Could you check a few things on this model? Use its own coordinates, in mm. Face numbers are marked on the shaded views. A direction names the side the tool comes from. Coordinates: 2 decimals unless noted, no trailing zeros. Order: outer loops, then holes, each group sorted by start corner. A loop starts at its lowest first (then second) coordinate and runs counter-clockwise, first axis right, second up. Notation, with made-up numbers: (44, 38.25) -> (55, 38.25) arc R17 cw to (55, 44.25) -> close; hole circle Ø1 at (40.25, -9.75). An arc over 180 degrees is marked (long way). Put each result on its own line as item: value. Start each with the question number.
Q1. Please list where these lines run through material, in increasing order: line 1 along X through (y, z) = (25, 0); line 2 along Z through (x, y) = (0, 27); line 3 along Z through (x, y) = (32.5, 40).
Q2. If we section it at A-A (x = 0): Please give me the cut outline in (y, z).
Q3. We'd pull the mould along Z, two halves only. Please class the marked faces 1, 2 and 3: +Z half, -Z half, draft (parallel to the pull), parting line (faces both ways), or undercut.
Q4. Will these pins go through, and if not, where does the flat tip stop? pin 1 (7.5 mm diameter, centred on y = 50, z = 45, fed in from -X); pin 2 (24.5 mm diameter, centred on x = -38.5, z = -24, fed in from +Y); pin 3 (7.5 mm diameter, centred on y = 51.5, z = -38, fed in from +X); pin 4 (2 mm diameter, centred on y = 25, z = -28, fed in from +X).
Q5. For the marked faces 4, 5 and 6, which set-ups out of +Z, -Z, +X, -X, +Y, -Y let a thin tool reach every point of the face, with its end or its side?
Q6. If we section it at C-C (y = 19.5): Please give me the cut outline in (x, z), and give its area (3 significant figures).
Q7. If we section it at D-D (x = 45.5): Please give me the cut outline in (y, z).
Q8. If we section it at B-B (y = 44): Count the separate pieces of the cut face and the enclosed holes in it, and give its area (3 significant figures).
from build123d import *

# Parameters (mm, degrees)
HEX_BODY_104AF_X_60_DEPTH      = 60
CROWN_CHAMFER_SKETCH_OUTSIDE_W = 276.052
CROWN_CHAMFER_SKETCH_OUTSIDE_H = 259.964
CROWN_CHAMFER_SKETCH_OUTSIDE_R = 52
CROWN_CHAMFER_45DEG_DEPTH      = 60
CROWN_CHAMFER_45DEG_DRAFT      = -45
BORE_SKETCH_50_R               = 25
BORE_50_DEPTH                  = 60
CASTLE_SLOTS_6X10_DEPTH        = 25


with BuildPart() as part:
    # Hex Profile Sketch → Hex Body 104AF x 60 (new body)
    with BuildSketch(Plane(origin=(0, 0, 0), x_dir=(1, 0, 0), z_dir=(0, 1, 0))):
        Polygon((30.022213998, -52), (60.044427996, 0), (30.022213998, 52), (-30.022213998, 52), (-60.044427996, 0), (-30.022213998, -52), align=None)
    extrude(amount=HEX_BODY_104AF_X_60_DEPTH)


with BuildPart() as crown_chamfer_45deg_tool:
    # Crown Chamfer Sketch outside → Crown Chamfer 45deg (with draft: the straight prism first)
    with BuildSketch(Plane(origin=(0, 60, 0), x_dir=(1, 0, 0), z_dir=(0, 1, 0))):
        Rectangle(CROWN_CHAMFER_SKETCH_OUTSIDE_W, CROWN_CHAMFER_SKETCH_OUTSIDE_H)
        Circle(CROWN_CHAMFER_SKETCH_OUTSIDE_R, mode=Mode.SUBTRACT)
    extrude(amount=-CROWN_CHAMFER_45DEG_DEPTH)
    # Crown Chamfer 45deg: the draft: its side faces are tilted about the plane it starts from
    crown_chamfer_45deg_sides = [crown_chamfer_45deg_tool.faces().sort_by_distance(p)[0] for p in [
        (0, 30, 129.982),
        (138.026, 30, 0),
        (0, 30, -129.982),
        (-138.026, 30, 0),
        (-52, 30, 0),
    ]]
    draft(crown_chamfer_45deg_sides, Plane(origin=(0, 60, 0), x_dir=(1, 0, 0), z_dir=(0, 1, 0)), CROWN_CHAMFER_45DEG_DRAFT)


with BuildPart() as part_1:
    add(part.part)

    # Crown Chamfer 45deg: cut by crown_chamfer_45deg_tool
    add(crown_chamfer_45deg_tool.part, mode=Mode.SUBTRACT)

    # Bore Sketch Ø50 → Bore Ø50 (cut)
    with BuildSketch(Plane(origin=(0, 60, 0), x_dir=(1, 0, 0), z_dir=(0, 1, 0))):
        with Locations(Location((0, 0, 0), (0, 0, 270))):
            Circle(BORE_SKETCH_50_R)
    extrude(amount=-BORE_50_DEPTH, mode=Mode.SUBTRACT)

    # Castle Slots Sketch → Castle Slots 6x10 (cut)
    with BuildSketch(Plane(origin=(0, 60, 0), x_dir=(1, 0, 0), z_dir=(0, 1, 0))):
        with BuildLine():
            Line((-5, -24.494897428), (-5, -52))
            Line((-5, -52), (0, -52))
            Line((0, -52), (5, -52))
            Line((5, -52), (5, -24.494897428))
            ThreePointArc((5, -24.494897428), (0, -25), (-5, -24.494897428))
        make_face()
        with BuildLine():
            Line((-23.713203436, -7.917321695), (-47.533320997, -21.669872981))
            Line((-47.533320997, -21.669872981), (-45.033320997, -26))
            Line((-45.033320997, -26), (-42.533320997, -30.330127019))
            Line((-42.533320997, -30.330127019), (-18.713203436, -16.577575733))
            ThreePointArc((-18.713203436, -16.577575733), (-21.650635095, -12.5), (-23.713203436, -7.917321695))
        make_face()
        with BuildLine():
            Line((-18.713203436, 16.577575733), (-42.533320997, 30.330127019))
            Line((-42.533320997, 30.330127019), (-45.033320997, 26))
            Line((-45.033320997, 26), (-47.533320997, 21.669872981))
            Line((-47.533320997, 21.669872981), (-23.713203436, 7.917321695))
            ThreePointArc((-23.713203436, 7.917321695), (-21.650635095, 12.5), (-18.713203436, 16.577575733))
        make_face()
        with BuildLine():
            Line((5, 24.494897428), (5, 52))
            Line((5, 52), (0, 52))
            Line((0, 52), (-5, 52))
            Line((-5, 52), (-5, 24.494897428))
            ThreePointArc((-5, 24.494897428), (0, 25), (5, 24.494897428))
        make_face()
        with BuildLine():
            Line((23.713203436, 7.917321695), (47.533320997, 21.669872981))
            Line((47.533320997, 21.669872981), (45.033320997, 26))
            Line((45.033320997, 26), (42.533320997, 30.330127019))
            Line((42.533320997, 30.330127019), (18.713203436, 16.577575733))
            ThreePointArc((18.713203436, 16.577575733), (21.650635095, 12.5), (23.713203436, 7.917321695))
        make_face()
        with BuildLine():
            Line((18.713203436, -16.577575733), (42.533320997, -30.330127019))
            Line((42.533320997, -30.330127019), (45.033320997, -26))
            Line((45.033320997, -26), (47.533320997, -21.669872981))
            Line((47.533320997, -21.669872981), (23.713203436, -7.917321695))
            ThreePointArc((23.713203436, -7.917321695), (21.650635095, -12.5), (18.713203436, -16.577575733))
        make_face()
    extrude(amount=-CASTLE_SLOTS_6X10_DEPTH, mode=Mode.SUBTRACT)


solid = part_1.part
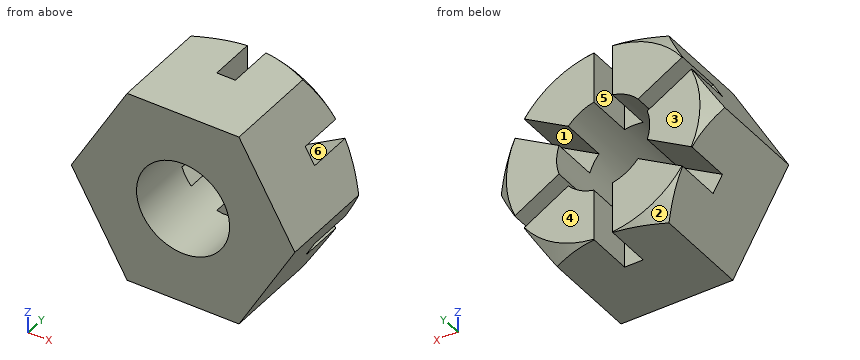
The answers:
1. line 1: -60.04 to -25, 25 to 60.04
1. line 2: -52 to -25, 25 to 52
1. line 3: -47.71 to -24.54, -12.99 to 12.99, 24.54 to 47.71
2. outline: (0, -52) -> (35, -52) -> (35, -25) -> (0, -25) -> close; (0, 25) -> (35, 25) -> (35, 52) -> (0, 52) -> close
3. face 1: undercut
3. face 2: -Z half
3. face 3: draft
4. pin 1: x = -36.23
4. pin 2: y = 60
4. pin 3: x = 40.27
4. pin 4: x = 44.46
5. face 4: +Z, -Z, +X, -X, +Y
5. face 5: +Z, -Z, +Y
5. face 6: +Y
6. outline: (-60.04, 0) -> (-30.02, -52) -> (30.02, -52) -> (60.04, 0) -> (30.02, 52) -> (-30.02, 52) -> close; hole circle Ø50 at (0, 0)
6. area: 7,400 mm^2
7. outline: (0, -25.19) -> (35, -25.19) -> (35, -20.5) -> (60, -20.5) -> (60, 20.5) -> (35, 20.5) -> (35, 25.19) -> (0, 25.19) -> close
8. separate pieces: 6
8. enclosed holes: 0
8. area: 5,770 mm^2
